The drawing under review shows one solid part. Ordinate dimensions are in mm from its lowest x, y, z. A direction names the side the tool comes from. Coordinates: 2 decimals unless noted, no trailing zeros. Write each loop counter-clockwise with the first axis right and the second up, starting at its lowest first coordinate (ties: lowest second). Pieces come first, ordered by that corner, then holes.
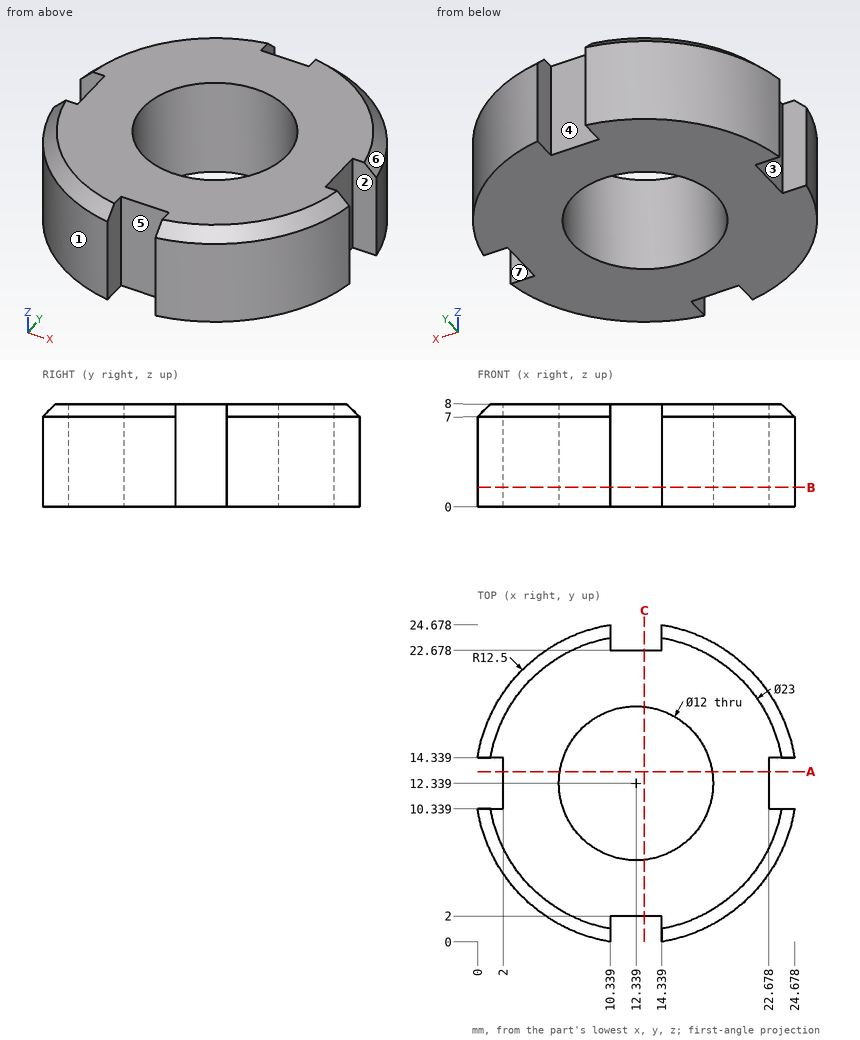
Q1. Add section B-B (z = 1.5). State the section outline as (x, y) points.
Ans:
outline: (0, 10.34) arc R12.5 ccw to (10.34, 0) - (10.34, 2) - (14.34, 2) - (14.34, 0) arc R12.5 ccw to (24.68, 10.34) - (22.68, 10.34) - (22.68, 14.34) - (24.68, 14.34) arc R12.5 ccw to (14.34, 24.68) - (14.34, 22.68) - (10.34, 22.68) - (10.34, 24.68) arc R12.5 ccw to (0, 14.34) - (2, 14.34) - (2, 10.34) - close; hole circle Ø12 at (12.34, 12.34)
Q2. Clearance check with flat-ended pins moving along their axes: pin 1 Ø4 at (x, z) = (19, 3) entering from -Y; pin 2 Ø2 at (x, z) = (13, 3) entering from -Y; pin 3 Ø2 at (y, z) = (12.5, 5.5) entering from -X; pin 4 Ø12 at (x, y) = (22, 18) entering from -Z. State where each tip first meets the part, or that it passes through.
Ans:
pin 1: stops at y = 0.74
pin 2: stops at y = 2
pin 3: stops at x = 2
pin 4: stops at z = 0
Q3. Tool access review of the marked faces 1, 2 and 3: name each direction out of +Z, -Z, +X, -X, +Y, -Y from which nothing blocks a thin tool from reaching the whole face with its end or side.
Ans:
face 1: +Z, -Z, -X, -Y
face 2: +Z, -Z, +X
face 3: +Z, -Z, -X
Q4. For probe 1 along X at (y, z) = (10, 2.5); probe 2 along X at (y, z) = (12, 0.75); probe 3 along Y at (x, z) = (9, 6.5) (1 decimal), list the stretches that pass through material, from the lowest coordinate up.
Ans:
probe 1: x = 0.06 to 6.81, 17.86 to 24.62
probe 2: x = 2 to 6.35, 18.33 to 22.68
probe 3: y = 0.3 to 7.4, 17.3 to 24.4
Q5. Add section A-A (y = 13.25). State the section outline as (x, z) points, then the cut area to 3 significant figures.
Ans:
outline: (2, 0) - (6.41, 0) - (6.41, 8) - (2, 8) - close; (18.27, 0) - (22.68, 0) - (22.68, 8) - (18.27, 8) - close
area: 70.5 mm2
Q6. Draft analysis for pull direction X (two halves, no side actions). For the marked faces 4, 5, 6 and 7, state which applies: +X half, -X half, draft (parallel to the pull), parting line (faces both ways), or undercut.
Ans:
face 4: undercut
face 5: undercut
face 6: +X half
face 7: draft
Q7. Add section C-C (x = 13). State the section outline as (y, z) points.
Ans:
outline: (2, 0) - (6.38, 0) - (6.38, 8) - (2, 8) - close; (18.3, 0) - (22.68, 0) - (22.68, 8) - (18.3, 8) - close
